```python
from build123d import *

# Parameters (mm, degrees)
L_BRACKET_BASE_DEPTH      = 40
CORNER_BLOCK_DEPTH        = 7
UPRIGHT_ROUNDED_TOP_DEPTH = 7
HUB_SKETCH_30_R           = 15
HUB_30_DEPTH              = 18
BORE_SKETCH_22_R          = 11
BORE_22_DEPTH             = 18
RIB_1_DEPTH               = 12
RIB_2_DEPTH               = 12
TRIANGULAR_CUT_1_DEPTH    = 6
TRIANGULAR_CUT_2_DEPTH    = 6


with BuildPart() as part:
    # L Profile Sketch → L Bracket Base (new body)
    with BuildSketch(Plane.XY):
        Polygon((0, 0), (34, 0), (34, 60), (27, 60), (27, 7), (0, 7), align=None)
    extrude(amount=L_BRACKET_BASE_DEPTH)

    # Corner Block Sketch → Corner Block (add)
    with BuildSketch(Plane(origin=(0, 7, 0), x_dir=(1, 0, 0), z_dir=(0, 1, 0))):
        with BuildLine():
            Line((-5, -5), (-5, -35))
            ThreePointArc((-5, -35), (-3.535533906, -38.535533906), (0, -40))
            Line((0, -40), (0, 0))
            ThreePointArc((0, 0), (-3.535533906, -1.464466094), (-5, -5))
        make_face()
    extrude(amount=-CORNER_BLOCK_DEPTH)

    # Upright Top Arc Sketch → Upright Rounded Top (add)
    with BuildSketch(Plane.ZY.offset(-27)):
        with BuildLine():
            Line((0, 60), (40, 60))
            ThreePointArc((40, 60), (20, 80), (0, 60))
        make_face()
    extrude(amount=-UPRIGHT_ROUNDED_TOP_DEPTH)

    # Hub Sketch Ø30 → Hub Ø30 (add)
    with BuildSketch(Plane.ZY.offset(-27)):
        with Locations(Location((20, 60, 0), (0, 0, 180))):
            Circle(HUB_SKETCH_30_R)
    extrude(amount=HUB_30_DEPTH)

    # Bore Sketch Ø22 → Bore Ø22 (cut)
    with BuildSketch(Plane.ZY.offset(-9)):
        with Locations((20, 60)):
            Circle(BORE_SKETCH_22_R)
    extrude(amount=-BORE_22_DEPTH, mode=Mode.SUBTRACT)

    # Rib 1 Sketch → Rib 1 (add)
    with BuildSketch(Plane.XY.offset(40)):
        Polygon((27, 7), (27, 27), (7, 7), align=None)
    extrude(amount=-RIB_1_DEPTH)

    # Rib 2 Sketch → Rib 2 (add)
    with BuildSketch(Plane(origin=(0, 0, 0), x_dir=(-1, 0, 0), z_dir=(0, 0, -1))):
        Polygon((-27, 7), (-7, 7), (-27, 27), align=None)
    extrude(amount=-RIB_2_DEPTH)

    # Triangular Cut 1 Sketch → Triangular Cut 1 (cut)
    with BuildSketch(Plane(origin=(0, 0, 0), x_dir=(-1, 0, 0), z_dir=(0, 0, -1))):
        Polygon((-27, 27), (-7, 7), (-27, 7), align=None)
    extrude(amount=-TRIANGULAR_CUT_1_DEPTH, mode=Mode.SUBTRACT)

    # Triangular Cut 2 Sketch → Triangular Cut 2 (cut)
    with BuildSketch(Plane.XY.offset(40)):
        Polygon((27, 27), (7, 7), (27, 7), align=None)
    extrude(amount=-TRIANGULAR_CUT_2_DEPTH, mode=Mode.SUBTRACT)


solid = part.part
```
CAD build for the part. Positions are in the model's coordinates, mm. A direction names the side the tool comes from. Coordinates: 2 decimals unless noted, no trailing zeros. Write each loop counter-clockwise with the first axis right and the second up, starting at its lowest first coordinate (ties: lowest second). Pieces come first, ordered by that corner, then holes.
(1) Cut at A-A, the plane x = 16.5. List the corners of the cut face in (y, z), and give its area (3 significant figures).
(2) Flat gauge pins, fed straight in: pin 1 (10 mm diameter, centred on x = 12.5, y = 13, fed in from +Z); pin 2 (10 mm diameter, centred on x = 13, y = 21, fed in from -Z); pin 3 (9 mm diameter, centred on y = 67, z = 16.5, fed in from -X); pin 4 (5 mm diameter, centred on x = 20, y = 60, fed in from -Z). Where does each tip first touch, or does it go through?
(3) Cut at C-C, the plane x = 12. List the corners of the cut face in (y, z).
(4) Cut at D-D, the plane y = 56.5. List the corners of the cut face in (x, z), and give its area (3 significant figures).
(5) Two-plate mould, pull along Z, no slides. Class faces 5 (the face through (27.2, 23.5, 0)), 6 (the face through (28, 23, 40)), 7 (the face through (7, 7, 20)), 8 (the face through (-5, 4, 20)): +Z half, -Z half, draft (parallel to the pull), parting line (faces both ways), or undercut.
(6) Drill centre lines: probe 1 along Y at (x, z) = (21.5, 20); probe 2 along Z at (x, y) = (15, 14.5); probe 3 along Y at (x, z) = (21, 12.5). Where is each one in solid material? Low to high.
(7) Cut at B-B, the plane z = 20. List the corners of the cut face in (x, y), and give its area (3 significant figures).
(8) 3-axis set-ups, long thin cutter, end or side, ignore diameter. For faces 1 (the face through (27, 60, 20)), 2 (the face through (21, 13, 34)), 3 (the face through (9, 50, 25)), 4 (the face through (21, 13, 6)): which of +Z, -Z, +X, -X, +Y, -Y reach the whole face in a straight line?
Geometry says:
1. outline: (0, 0) - (7, 0) - (7, 6) - (16.5, 6) - (16.5, 12) - (7, 12) - (7, 28) - (16.5, 28) - (16.5, 34) - (7, 34) - (7, 40) - (0, 40) - close; circle Ø30 at (60, 20); hole circle Ø22 at (60, 20)
1. area: 721 mm2
2. pin 1: stops at z = 34
2. pin 2: passes through
2. pin 3: stops at x = 9
2. pin 4: stops at z = 5
3. outline: (0, 0) - (7, 0) - (7, 6) - (12, 6) - (12, 12) - (7, 12) - (7, 28) - (12, 28) - (12, 34) - (7, 34) - (7, 40) - (0, 40) - close; circle Ø30 at (60, 20); hole circle Ø22 at (60, 20)
4. outline: (9, 5.41) - (27, 5.41) - (27, 0) - (34, 0) - (34, 40) - (27, 40) - (27, 34.59) - (9, 34.59) - (9, 30.43) - (27, 30.43) - (27, 9.57) - (9, 9.57) - close
4. area: 430 mm2
5. face 5: -Z half
5. face 6: +Z half
5. face 7: undercut
5. face 8: draft
6. probe 1: y = 0 to 7, 45 to 49, 71 to 75
6. probe 2: z = 6 to 12, 28 to 34
6. probe 3: y = 0 to 7, 47.01 to 51.95, 68.05 to 72.99
7. outline: (-5, 0) - (34, 0) - (34, 80) - (27, 80) - (27, 75) - (9, 75) - (9, 71) - (27, 71) - (27, 49) - (9, 49) - (9, 45) - (27, 45) - (27, 7) - (-5, 7) - close
7. area: 928 mm2
8. face 1: -X
8. face 2: +Z, -X
8. face 3: +Z, -Z, -X, +Y
8. face 4: -Z, -X
